```python
from build123d import *

# Parameters (mm, degrees)
SKETCH_1_W          = 200.3
SKETCH_1_H          = 146.3
EXTRUDE_1_DEPTH     = 6
SKETCH_2_W          = 189.6
SKETCH_2_H          = 135.6
EXTRUDE_2_DEPTH     = 28
SKETCH_3_W          = 188.3
SKETCH_3_H          = 134.3
CUT_EXTRUDE_1_DEPTH = 1


with BuildPart() as part:
    # 草图1 → 凸台-拉伸1 (new body)
    with BuildSketch(Plane.XY):
        Rectangle(SKETCH_1_W, SKETCH_1_H)
    extrude(amount=EXTRUDE_1_DEPTH)

    # 草图2 → 凸台-拉伸2 (add)
    with BuildSketch(Plane(origin=(0, 0, 0), x_dir=(-1, 0, 0), z_dir=(0, 0, -1))):
        Rectangle(SKETCH_2_W, SKETCH_2_H)
    extrude(amount=EXTRUDE_2_DEPTH)

    # 草图3 → 切除-拉伸1 (cut)
    with BuildSketch(Plane.XY.offset(6)):
        Rectangle(SKETCH_3_W, SKETCH_3_H)
    extrude(amount=-CUT_EXTRUDE_1_DEPTH, mode=Mode.SUBTRACT)


solid = part.part
```
Geometry: final body of the model. Coordinates: model frame, mm. A direction names the side the tool comes from. Coordinates: 2 decimals unless noted, no trailing zeros. Order: outer loops, then holes, each group sorted by start corner. A loop starts at its lowest first (then second) coordinate and runs counter-clockwise, first axis right, second up.
Item 1: Contact query for flat-ended pins moving along their axis: P1, Ø14, axis at y = 1.5, z = -12, coming from the -X side; P2, Ø3, axis at x = 72.5, z = -4.5, coming from the -Y side; P3, Ø12, axis at x = -38, y = 49.5, coming from the +Z side. Output: stop coordinate, or through.
Answer:
P1: stops at x = -94.8
P2: stops at y = -67.8
P3: stops at z = 5
Item 2: Material intervals for line 1 along Y through (x, z) = (66.5, -11.5); line 2 along X through (y, z) = (-25, -21); line 3 along Z through (x, y) = (34, -6.5), sorted ascending.
Answer:
line 1: y = -67.8 to 67.8
line 2: x = -94.8 to 94.8
line 3: z = -28 to 5
Item 3: Section query C-C (z = -16). Output: boundary loops of the cut face in (x, y), then the cut area to 3 significant figures.
Answer:
outline: (-94.8, -67.8) - (94.8, -67.8) - (94.8, 67.8) - (-94.8, 67.8) - close
area: 25,700 mm2
Item 4: Section query A-A (x = -15.5). Output: boundary loops of the cut face in (y, z).
Answer:
outline: (-73.15, 0) - (-67.8, 0) - (-67.8, -28) - (67.8, -28) - (67.8, 0) - (73.15, 0) - (73.15, 6) - (67.15, 6) - (67.15, 5) - (-67.15, 5) - (-67.15, 6) - (-73.15, 6) - close
Item 5: Access query for faces 5 (the face through (-1, 73.15, 3)), 6 (the face through (1, 67.8, -14)). Directions: +Z, -Z, +X, -X, +Y, -Y. A direction counts if a zero-diameter tool reaches every point of the face in a straight line with its end or side. Return the directions, or none.
Answer:
face 5: +Z, -Z, +X, -X, +Y
face 6: -Z, +X, -X, +Y
Item 6: Section query B-B (y = -41.5). Output: boundary loops of the cut face in (x, z).
Answer:
outline: (-100.15, 0) - (-94.8, 0) - (-94.8, -28) - (94.8, -28) - (94.8, 0) - (100.15, 0) - (100.15, 6) - (94.15, 6) - (94.15, 5) - (-94.15, 5) - (-94.15, 6) - (-100.15, 6) - close
Item 7: Draft query along X for faces 1 (the face through (-94.8, -1, -14)), 2 (the face through (1, -67.8, -14)), 3 (the face through (-1, 1, 5)), 4 (the face through (94.8, -1, -14)). Return one class per face: released by +X, released by -X, zero draft, split by the parting line, or undercut.
Answer:
face 1: released by -X
face 2: zero draft
face 3: undercut
face 4: released by +X
